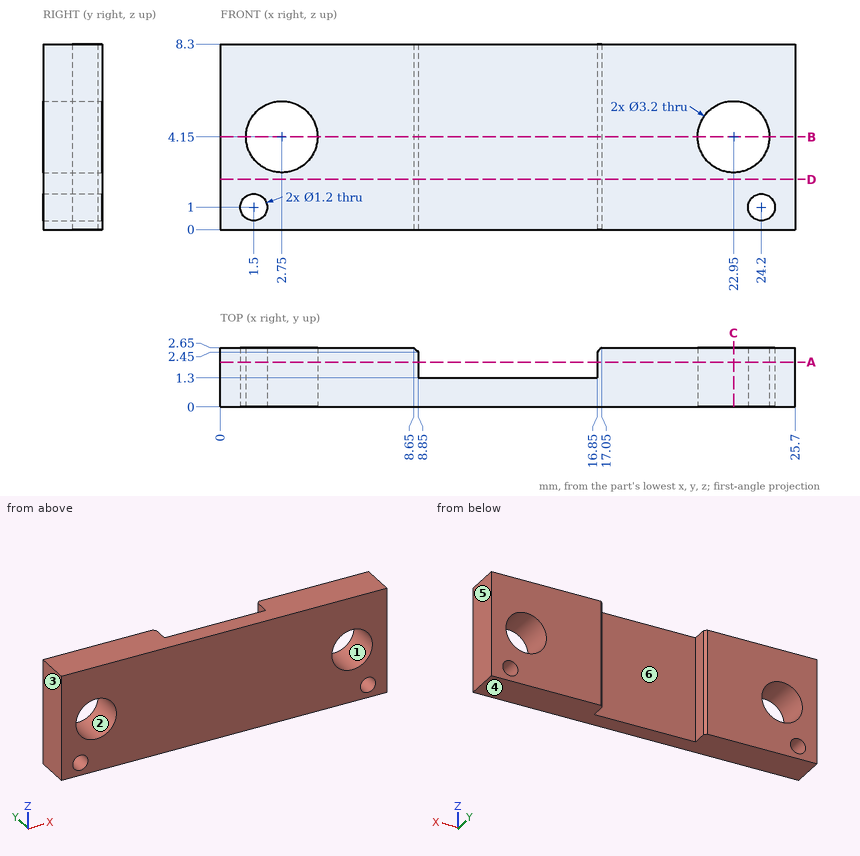
Part print with two shaded views. Sizes in mm from the minimum x, y, z corner. A direction names the side the tool comes from. Give positions to 0.01 mm unless a question says otherwise; leave off trailing zeros. Write each loop counter-clockwise with the first axis right and the second up, starting at its lowest first coordinate (ties: lowest second). Pieces come first, ordered by that corner, then holes.
1) Which spindle directions (+Z, -Z, +X, -X, +Y, -Y) get a long thin tool onto all of the face, cutting with end or side? Do the marked faces 5 and 6. Say none if no direction does.
Resolved:
face 5: +Z, -Z, +X, +Y, -Y
face 6: +Z, -Z, +Y
2) Cut at A-A on y = 2. Write the cut outline in (x, z), then the cut area to 3 significant figures.
Resolved:
outline: (0, 0) - (8.85, 0) - (8.85, 8.3) - (0, 8.3) - close; (16.85, 0) - (25.7, 0) - (25.7, 8.3) - (16.85, 8.3) - close; hole circle Ø1.2 at (1.5, 1); hole circle Ø3.2 at (2.75, 4.15); hole circle Ø3.2 at (22.95, 4.15); hole circle Ø1.2 at (24.2, 1)
area: 129 mm2
3) Cut at C-C on x = 22.95. Write the cut outline in (y, z).
Resolved:
outline: (0, 0) - (2.65, 0) - (2.65, 2.55) - (0, 2.55) - close; (0, 5.75) - (2.65, 5.75) - (2.65, 8.3) - (0, 8.3) - close
4) Cut at D-D on z = 2.25. Write the cut outline in (x, y), then the cut area to 3 significant figures.
Resolved:
outline: (0, 0) - (25.7, 0) - (25.7, 2.65) - (17.05, 2.65) - (16.85, 2.45) - (16.85, 1.3) - (8.85, 1.3) - (8.85, 2.45) - (8.65, 2.65) - (0, 2.65) - close
area: 57.3 mm2
5) Two-plate mould, pull along Z, no slides. Class the marked faces 1, 2, 3 and 4: released by +Z, released by -Z, zero draft, split by the parting line, or undercut.
Resolved:
face 1: undercut
face 2: undercut
face 3: zero draft
face 4: released by -Z
6) Probe L1, parallel to X at y = 2.15, z = 1; L2, parallel to X at y = 0.45, z = 4.25; L3, parallel to X at y = 2.05, z = 4.15. List the from-to ranges inside material, lowest first.
Resolved:
L1: x = 0 to 0.9, 2.1 to 8.85, 16.85 to 23.6, 24.8 to 25.7
L2: x = 0 to 1.15, 4.35 to 21.35, 24.55 to 25.7
L3: x = 0 to 1.15, 4.35 to 8.85, 16.85 to 21.35, 24.55 to 25.7
7) Cut at B-B on z = 4.15. Write the cut outline in (x, y), then the cut area to 3 significant figures.
Resolved:
outline: (0, 0) - (1.15, 0) - (1.15, 2.65) - (0, 2.65) - close; (4.35, 0) - (21.35, 0) - (21.35, 2.65) - (17.05, 2.65) - (16.85, 2.45) - (16.85, 1.3) - (8.85, 1.3) - (8.85, 2.45) - (8.65, 2.65) - (4.35, 2.65) - close; (24.55, 0) - (25.7, 0) - (25.7, 2.65) - (24.55, 2.65) - close
area: 40.3 mm2
